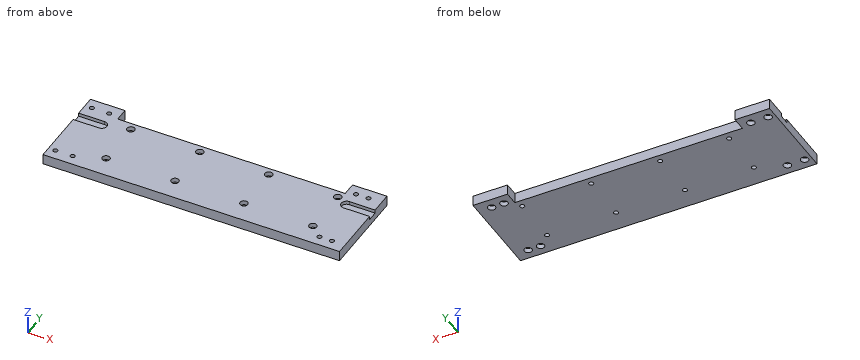
```python
from build123d import *

# Parameters (mm, degrees)
SKETCH1_W                                            = 430
SKETCH1_H                                            = 130
BOSS_EXTRUDE1_DEPTH                                  = 15
HOLE_SIZE_PER_SOCKET_HEAD_CAP_SCREW_TYPE_D           = 6.6
HOLE_SIZE_PER_SOCKET_HEAD_CAP_SCREW_TYPE_CBORE_D     = 11
HOLE_SIZE_PER_SOCKET_HEAD_CAP_SCREW_TYPE_CBORE_DEPTH = 6.8
CUT_EXTRUDE1_DEPTH                                   = 5
CBORE_FOR_M6_HEX_SOCKET_HEAD_CAP_SCREW1_D            = 6.6
CBORE_FOR_M6_HEX_SOCKET_HEAD_CAP_SCREW1_CBORE_D      = 11
CBORE_FOR_M6_HEX_SOCKET_HEAD_CAP_SCREW1_CBORE_DEPTH  = 6.4
SKETCH8_W                                            = 330
SKETCH8_H                                            = 15
CUT_EXTRUDE2_DEPTH                                   = 20


with BuildPart() as part:
    # Sketch1 → Boss-Extrude1 (new body)
    with BuildSketch(Plane.XY):
        with Locations((215, 65)):
            Rectangle(SKETCH1_W, SKETCH1_H)
    extrude(amount=BOSS_EXTRUDE1_DEPTH)

    # Hole size per socket head cap screw type 0 (through all)
    with Locations(Plane(origin=(0, 0, 0), x_dir=(-1, 0, 0), z_dir=(0, 0, -1))):
        with Locations((-10, 15), (-10, 115), (-35, 15), (-35, 115), (-393, 15), (-411, 15), (-393, 115), (-411, 115)):
            CounterBoreHole(HOLE_SIZE_PER_SOCKET_HEAD_CAP_SCREW_TYPE_D / 2, HOLE_SIZE_PER_SOCKET_HEAD_CAP_SCREW_TYPE_CBORE_D / 2, HOLE_SIZE_PER_SOCKET_HEAD_CAP_SCREW_TYPE_CBORE_DEPTH)

    # Sketch5 → Cut-Extrude1 (cut)
    with BuildSketch(Plane.XY.offset(15)):
        with BuildLine():
            Line((430, 97.5), (430, 82.5))
            Line((430, 82.5), (392.5, 82.5))
            ThreePointArc((392.5, 82.5), (385, 90), (392.5, 97.5))
            Line((392.5, 97.5), (430, 97.5))
        make_face()
        with BuildLine():
            Line((37.5, 82.5), (0, 82.5))
            Line((0, 82.5), (0, 97.5))
            Line((0, 97.5), (37.5, 97.5))
            ThreePointArc((37.5, 97.5), (45, 90), (37.5, 82.5))
        make_face()
    extrude(amount=-CUT_EXTRUDE1_DEPTH, mode=Mode.SUBTRACT)

    # CBORE for M6 Hex Socket Head Cap Screw1 (through all)
    with Locations(Plane.XY.offset(15)):
        with Locations((75, 99), (175, 99), (75, 31), (175, 31), (275, 99), (275, 31), (375, 99), (375, 31)):
            CounterBoreHole(CBORE_FOR_M6_HEX_SOCKET_HEAD_CAP_SCREW1_D / 2, CBORE_FOR_M6_HEX_SOCKET_HEAD_CAP_SCREW1_CBORE_D / 2, CBORE_FOR_M6_HEX_SOCKET_HEAD_CAP_SCREW1_CBORE_DEPTH)

    # Sketch8 → Cut-Extrude2 (cut)
    with BuildSketch(Plane(origin=(0, 130, 0), x_dir=(1, 0, 0), z_dir=(0, 1, 0))):
        with Locations((215, -7.5)):
            Rectangle(SKETCH8_W, SKETCH8_H)
    extrude(amount=-CUT_EXTRUDE2_DEPTH, mode=Mode.SUBTRACT)


solid = part.part
```
Design review of the part built by this model. Coordinates are the model's own, in mm. Give positions to 0.01 mm unless a question says otherwise; leave off trailing zeros. Write each loop counter-clockwise with the first axis right and the second up, starting at its lowest first coordinate (ties: lowest second). Pieces come first, ordered by that corner, then holes.
(1) Clearance check with flat-ended pins moving along their axes: pin 1 Ø2 at (x, z) = (271, 12) entering from +Y; pin 2 Ø5.5 at (x, y) = (275, 29) entering from +Z; pin 3 Ø4.5 at (x, y) = (415, 89.5) entering from +Z; pin 4 Ø6.5 at (x, y) = (275, 99) entering from +Z. State where each tip first meets the part, or that it passes through.
Checked values:
pin 1: stops at y = 110
pin 2: stops at z = 8.6
pin 3: stops at z = 10
pin 4: passes through
(2) Wall thickness on line 1 along Y through (x, z) = (375, 5.5); line 2 along Y through (x, z) = (75, 13.75); line 3 along X through (y, z) = (33, 11.5): over which ranges is each line inside the solid? List them lowest first.
Checked values:
line 1: y = 0 to 27.7, 34.3 to 95.7, 102.3 to 110
line 2: y = 0 to 25.5, 36.5 to 93.5, 104.5 to 110
line 3: x = 0 to 69.88, 80.12 to 169.88, 180.12 to 269.88, 280.12 to 369.88, 380.12 to 430
(3) Add section A-A (x = 117). Give the boundary of the cut face in (y, z).
Checked values:
outline: (0, 0) - (110, 0) - (110, 15) - (0, 15) - close
